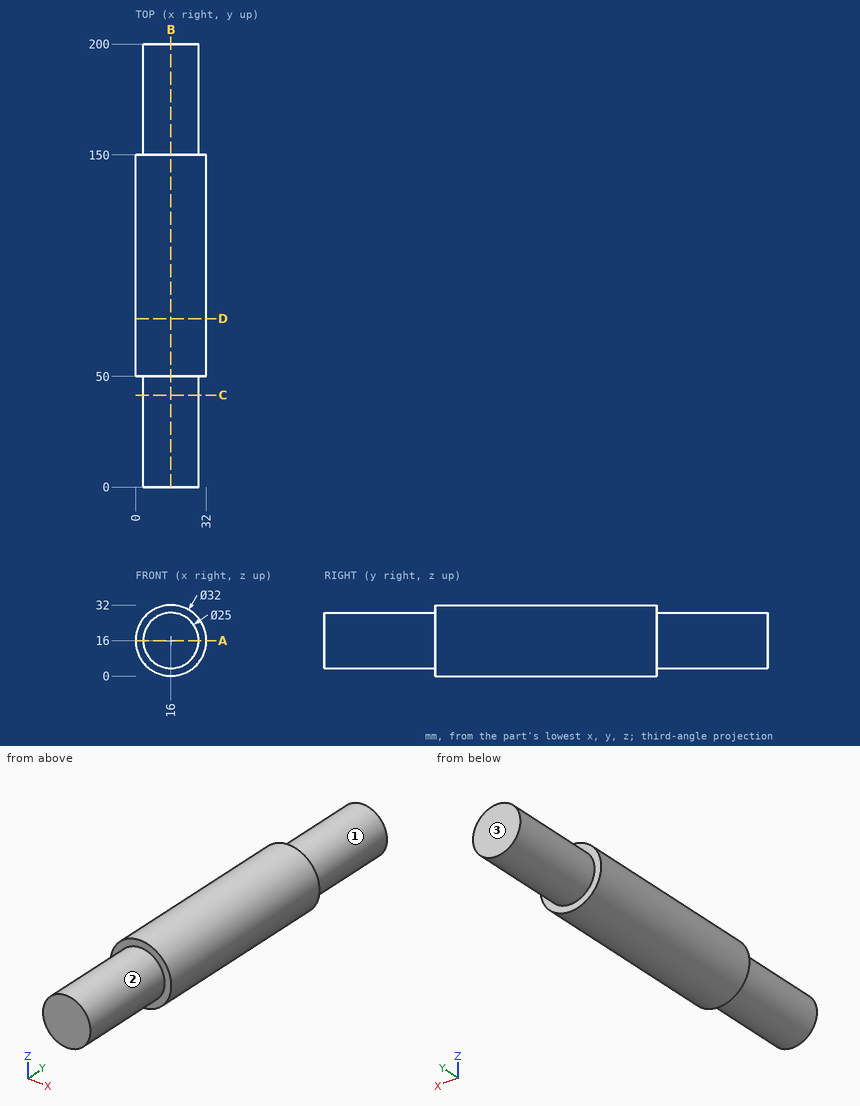
Can you work these out from the drawing? Everything is in mm from the part's minimum corner. A direction names the side the tool comes from. Give positions to 0.01 mm unless a question says otherwise; leave off trailing zeros. Loops run counter-clockwise (first coordinate to the right, second up) from the corner with the lowest first, then second, coordinate; pieces in that order, holes last. Notation, with made-up numbers: (41, 36.5) -> (51, 36.5) arc R28 cw to (51, 59.5) -> close; hole circle Ø5 at (-19.75, -27). An arc over 180 degrees is marked (long way). Write item = value, one per line.
1) For the marked faces 1, 2 and 3, which set-ups out of +Z, -Z, +X, -X, +Y, -Y let a thin tool reach every point of the face, with its end or its side?
Check result:
face_1 = +Y
face_2 = -Y
face_3 = +Z, -Z, +X, -X, +Y
2) Suppose I cut it at B-B on x = 16. Write out the boundary of the cut face in (y, z), then the cut area to 3 significant figures.
Check result:
outline = (0, 3.5) -> (50, 3.5) -> (50, 0) -> (150, 0) -> (150, 3.5) -> (200, 3.5) -> (200, 28.5) -> (150, 28.5) -> (150, 32) -> (50, 32) -> (50, 28.5) -> (0, 28.5) -> close
area = 5,700 mm2
3) I need wall thicknesses on L1, parallel to Y at x = 8.5, z = 27.5; L2, parallel to Z at x = 4, y = 126; L3, parallel to Z at x = 25.5, y = 83. Which ranges of each line are inside material? Lowest first, please. Write a range as from..to.
Check result:
L1 = 50..150
L2 = 5.42..26.58
L3 = 3.13..28.87
4) Suppose I cut it at A-A on z = 16. Write out the boundary of the cut face in (x, y), then the cut area to 3 significant figures.
Check result:
outline = (0, 50) -> (3.5, 50) -> (3.5, 0) -> (28.5, 0) -> (28.5, 50) -> (32, 50) -> (32, 150) -> (28.5, 150) -> (28.5, 200) -> (3.5, 200) -> (3.5, 150) -> (0, 150) -> close
area = 5,700 mm2
5) Will these pins go through, and if not, where does the flat tip stop? pin 1 (2 mm diameter, centred on x = 18, y = 74.5, fed in from +Z); pin 2 (8 mm diameter, centred on x = 7, y = 102.5, fed in from -Z); pin 3 (4 mm diameter, centred on y = 135.5, z = 12, fed in from -X).
Check result:
pin_1 = 31.97
pin_2 = 0.8
pin_3 = 0.13
6) Suppose I cut it at C-C on y = 41.5. Write out the boundary of the cut face in (x, z), then the cut area to 3 significant figures.
Check result:
outline = circle Ø25 at (16, 16)
area = 491 mm2
7) Suppose I cut it at D-D on y = 76. Write out the boundary of the cut face in (x, z), then the cut area to 3 significant figures.
Check result:
outline = circle Ø32 at (16, 16)
area = 804 mm2
